```python
from build123d import *

# Parameters (mm, degrees)
CUT_EXTRUDE_1_DEPTH      = 312.287648325
CUT_EXTRUDE_1_DEPTH_BACK = 312.287648325
SKETCH_2_R               = 7
CHAMFER_1_SIZE           = 2
FILLET_1_R               = 7


with BuildPart() as part:
    # 草图1 → 旋转1 (revolve)
    with BuildSketch(Plane.XY, mode=Mode.PRIVATE) as revolve_1_sk:
        Polygon((0, 0), (0, 15), (27, 15), (27, 13), (31, 13), (31, 16), (36, 16), (36, 14.5), (38, 14.5), (38, 16), (43, 16), (43, 14.5), (45, 14.5), (45, 16), (50, 16), (50, 20), (260.669872981, 20), (270, 17.5), (310, 17.5), (310, 0), align=None)
    revolve(revolve_1_sk.sketch.rotate(Axis((0, 0, 0), (1, 0, 0)), 90), axis=Axis((0, 0, 0), (1, 0, 0)))

    # 草图2 → 切除-拉伸1 (cut, two sides: drawn at the far end of the back side and taken through both)
    with BuildSketch(Plane(origin=(0, 0, 0), x_dir=(1, 0, 0), z_dir=(0, 1, 0)).offset(-CUT_EXTRUDE_1_DEPTH_BACK)):
        with Locations(Location((290, 0, 0), (0, 0, 270))):
            Circle(SKETCH_2_R)
    extrude(amount=CUT_EXTRUDE_1_DEPTH + CUT_EXTRUDE_1_DEPTH_BACK, mode=Mode.SUBTRACT)

    # 倒角1
    chamfer_1_edges = [part.edges().sort_by_distance(p)[0] for p in [
        (0, 0, -15),
    ]]
    chamfer(chamfer_1_edges, length=CHAMFER_1_SIZE)

    # 圆角1
    fillet_1_edges = [part.edges().sort_by_distance(p)[0] for p in [
        (310, 0, -17.5),
    ]]
    fillet(fillet_1_edges, radius=FILLET_1_R)


solid = part.part
```
Input: part model. Units: mm. Frame: model coordinates. A direction names the side the tool comes from. Give positions to 0.01 mm unless a question says otherwise; leave off trailing zeros. Order: outer loops, then holes, each group sorted by start corner. A loop starts at its lowest first (then second) coordinate and runs counter-clockwise, first axis right, second up. Notation, with made-up numbers: (-39, 51.5) -> (0, 51.5) arc R21 ccw to (0, 63.5) -> close; hole circle Ø7 at (-25.75, -11). An arc over 180 degrees is marked (long way). Write each question's results on one line, items separated by ' | '. Start each with the question number.
Item 1: Contact query for flat-ended pins moving along their axis: P1, Ø12, axis at x = 229, y = -8, coming from the -Z side; P2, Ø11, axis at x = 290, z = 0, coming from the +Y side; P3, Ø2, axis at y = -12.5, z = 7, coming from the +X side; P4, Ø1.5, axis at x = 267.5, z = 4.5, coming from the -Y side. Output: stop coordinate, or through.
Item 2: Line query: line 1 (X direction, y = 6, z = 0); line 2 (X direction, y = 6, z = 5); line 3 (Z direction, x = 290, y = -4.5). Output: solid intervals per line, ascending.
Item 3: Mould query, pull axis X, two halves, no side actions, for faces 1 (the cylindrical face through (37.014, 12.864, 6.691)), 2 (the conical face through (0.125, 12.813, -2.845)), 3 (the cylindrical face through (14.68, -12.65, 8.06)). Classes: pulls with the +X half, pulls with the -X half, needs draft (parallel to the pull), parting line crosses it, or undercut.
Item 4: Cut plane B-B on x = 134.5. Return the cut outline in (y, z).
Item 5: Set-up query: faces 4 (the cylindrical face through (47.54, 15.62, -3.47)), 5 (the cylindrical face through (286.731, 6.703, 16.166)), 6 (the flat face through (36, -14.3, -3.6)), 7 (the flat face through (0, 0, 0)). Return all of +Z, -Z, +X, -X, +Y, -Y with unobstructed straight access to the full face (end or side cutting, diameter ignored); none if empty.
Item 6: Cut plane A-A on x = 290. Return the cut outline in (y, z).
Established:
1) P1: z = -19.9 | P2: through | P3: x = 309.4 | P4: y = -17.88
2) line 1: 0 to 283, 297 to 310 | line 2: 0 to 285.1, 294.9 to 310 | line 3: -16.91 to -7, 7 to 16.91
3) face 1: undercut | face 2: pulls with the -X half | face 3: needs draft
4) outline: circle Ø40 at (0, 0)
5) face 4: -X | face 5: +X | face 6: none | face 7: +Z, -Z, -X, +Y, -Y
6) outline: (-16.04, -7) arc R17.5 ccw to (16.04, -7) -> close; (-16.04, 7) -> (16.04, 7) arc R17.5 ccw to start
